Geometry check sheet. Reference: the model listing, model coordinates, mm. Round coordinates to 2 decimals unless told otherwise and drop trailing zeros. Order: outer loops, then holes, each group sorted by start corner. A loop starts at its lowest first (then second) coordinate and runs counter-clockwise, first axis right, second up. Notation, with made-up numbers: M -23.5,-9 L -18.5,-9 A25 cw -18.5,7 Z; hole C 46,61 d3. An arc over 180 degrees is marked long. Answer as a JSON object with one key per item and string values. Group by question number.
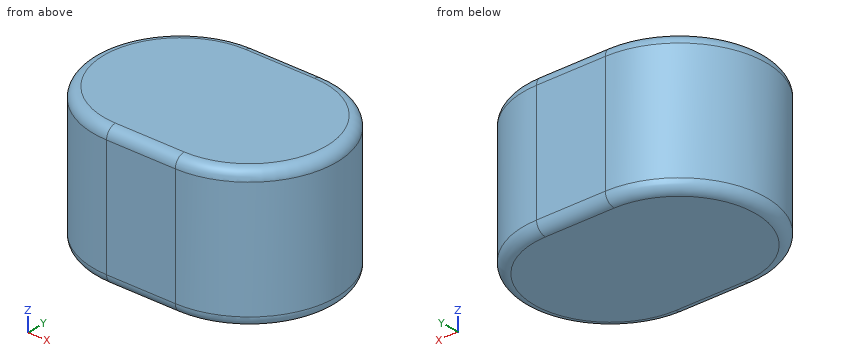
```python
from build123d import *

# Parameters (mm, degrees)
EXTRUDE_523_DEPTH = 8
FILLET_1_R        = 0.6


with BuildPart() as part:
    # 草图1 → Extrude 523 (new body)
    with BuildSketch(Plane.XY):
        with BuildLine():
            Line((-2, 5), (2, 5))
            ThreePointArc((2, 5), (7, 0), (2, -5))
            Line((2, -5), (-2, -5))
            ThreePointArc((-2, -5), (-7, 0), (-2, 5))
        make_face()
    extrude(amount=EXTRUDE_523_DEPTH)

    # 圆角1
    fillet_1_edges = [part.edges().sort_by_distance(p)[0] for p in [
        (7, 0, 8),
        (0, 5, 8),
        (-7, 0, 8),
        (0, 5, 0),
        (7, 0, 0),
        (0, -5, 0),
        (-7, 0, 0),
        (0, -5, 8),
    ]]
    fillet(fillet_1_edges, radius=FILLET_1_R)


solid = part.part
```
1) Go/stop test with flat-tipped pins: P1, Ø1.5, axis at y = 1.5, z = 6, coming from the -X side; P2, Ø4, axis at y = -2.5, z = 3.5, coming from the +X side. Record where each tip stops, or that it passes through.
2) Thickness scan on line 1 along X through (y, z) = (-4, 5.5); line 2 along Y through (x, z) = (-5.75, 0.75); line 3 along X through (y, z) = (-3, 2.25). Record the ranges inside material, lowest first. Write a range as [from, to].
3) Sectioned sample at A-A (z = 5.5). Record the boundary of the cut face in (x, y), then the cut area to 3 significant figures.
Final values:
{
 "1": {"P1": "stops at x = -6.94", "P2": "stops at x = 6.97"},
 "2": {"line 1": "x = [-5, 5]", "line 2": "y = [-3.31, 3.31]", "line 3": "x = [-6, 6]"},
 "3": {"outline": "M -2,-5 L 2,-5 A5 ccw 2,5 L -2,5 A5 ccw Z", "area": "119 mm^2"}
}
